from build123d import *

# Parameters (mm, degrees)
EXTRUDE_1_DEPTH = 150


with BuildPart() as part:
    # 草图1 → 凸台-拉伸1 (new body)
    with BuildSketch(Plane(origin=(0, 0, 0), x_dir=(1, 0, 0), z_dir=(0, 1, 0))):
        Polygon((0, 0), (130, 0), (130, 150), (60, 150), (60, 180), (10, 180), (10, 150), (0, 150), align=None)
    extrude(amount=EXTRUDE_1_DEPTH)


solid = part.part
Can you work these out from the model? Positions are in its coordinate system, mm. A direction names the side the tool comes from. Give positions to 0.01 mm unless a question says otherwise; leave off trailing zeros. Loops run counter-clockwise (first coordinate to the right, second up) from the corner with the lowest first, then second, coordinate; pieces in that order, holes last. Notation, with made-up numbers: (23.5, -31.5) - (44.5, -31.5) arc R25 ccw to (44.5, -18.5) - close; hole circle Ø8 at (9, 51). An arc over 180 degrees is marked (long way). Answer as a JSON object with one key per item and string values.
Q1. Imagine slicing it at A-A on y = 37. Write out the boundary of the cut face in (x, z), plus the area to 3 significant figures.
Geometry says:
{"outline": "(0, -150) - (10, -150) - (10, -180) - (60, -180) - (60, -150) - (130, -150) - (130, 0) - (0, 0) - close", "area": "21,000 mm²"}
Q2. Which directions (+Z, -Z, +X, -X, +Y, -Y) give clear straight access to the entire face, cutting with the end or side of a thin tool? Please do faces 1 (the flat face through (60, 74, -165)), 2 (the flat face through (0, 74, -76)), 3 (the flat face through (10, 74, -165)).
Geometry says:
{"face 1": "-Z, +X, +Y, -Y", "face 2": "+Z, -Z, -X, +Y, -Y", "face 3": "-Z, -X, +Y, -Y"}
Q3. If I drill on L1, parallel to X at y = 95.5, z = -172; L2, parallel to Z at x = 72.5, y = 16.5, over which ranges is the centre line in solid material (lowest first)?
Geometry says:
{"L1": "10 to 60", "L2": "-150 to 0"}
Q4. Will these pins go through, and if not, where does the flat tip stop? P1, Ø6, axis at x = 95.5, y = 115, coming from the +Z side; P2, Ø5, axis at y = 122.5, z = -155, coming from the -X side; P3, Ø15, axis at y = 93, z = -168.5, coming from the +X side.
Geometry says:
{"P1": "z = 0", "P2": "x = 10", "P3": "x = 60"}
Q5. Imagine slicing it at B-B on z = -159.5. Write out the boundary of the cut face in (x, y), plus the area to 3 significant figures.
Geometry says:
{"outline": "(10, 0) - (60, 0) - (60, 150) - (10, 150) - close", "area": "7,500 mm²"}
Q6. Imagine slicing it at C-C on x = 93. Write out the boundary of the cut face in (y, z).
Geometry says:
{"outline": "(0, -150) - (150, -150) - (150, 0) - (0, 0) - close"}
